For this review, use the dimensioned drawing (mm, ordinates from the lowest corner) and the shaded views. A direction names the side the tool comes from. Round coordinates to 2 decimals unless told otherwise and drop trailing zeros. Order: outer loops, then holes, each group sorted by start corner. A loop starts at its lowest first (then second) coordinate and runs counter-clockwise, first axis right, second up. Notation, with made-up numbers: M 47.5,-18.5 L 90.5,-18.5 A23 ccw 90.5,5.5 Z; hole C 31.25,36.5 d9. An arc over 180 degrees is marked long. One line per item, written item: value. Start each with the question number.
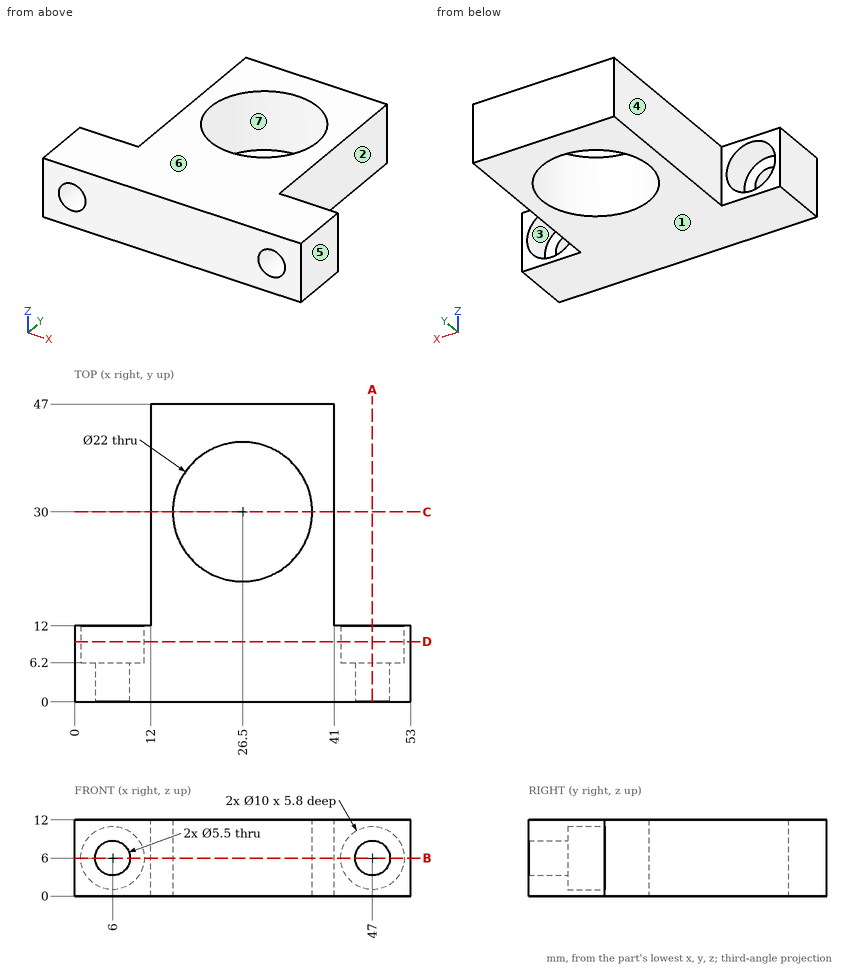
Item 1: The part is to be moulded in two halves that separate along X. For the marked faces 4, 5, 6 and 7, say which applies: pulls with the +X half, pulls with the -X half, needs draft (parallel to the pull), parting line crosses it, or undercut.
Item 2: Consider section A-A, the plane x = 47. Give the boundary of the cut face in (y, z), then the cut area to 3 significant figures.
Item 3: Machinability: for the marked faces 1, 2 and 3, which of the approach directions +Z, -Z, +X, -X, +Y, -Y give a long, thin tool a straight path to every point of the face, cutting with its end or side? Answer none if there is none.
Item 4: Consider section D-D, the plane y = 9.5. Give the boundary of the cut face in (x, z), then the cut area to 3 significant figures.
Item 5: Wall thickness on L1, parallel to Y at x = 26.5, z = 3; L2, parallel to Z at x = 47, y = 1.5; L3, parallel to X at y = 4, z = 8.25: over which ranges is each line inside the solid? List them lowest first.
Item 6: Consider section B-B, the plane z = 6. Give the boundary of the cut face in (x, y).
Item 7: Consider section C-C, the plane y = 30. Give the boundary of the cut face in (x, z), then the cut area to 3 significant figures.
Item 8: Clearance check with flat-ended pins moving along their axes: P1, Ø6, axis at x = 47, z = 6, coming from the -Y side; P2, Ø1.5, axis at x = 43.5, z = 9, coming from the +Y side; P3, Ø3.5, axis at x = 6, z = 6, coming from the +Y side (3 decimals); P4, Ø3.5, axis at y = 31, z = 7.5, coming from the +X side. State where each tip first meets the part, or that it passes through.
Computed:
1. face 4: pulls with the -X half
1. face 5: pulls with the +X half
1. face 6: needs draft
1. face 7: undercut
2. outline: M 0,0 L 12,0 L 12,1 L 6.2,1 L 6.2,3.25 L 0,3.25 Z; M 0,8.75 L 6.2,8.75 L 6.2,11 L 12,11 L 12,12 L 0,12 Z
2. area: 51.9 mm^2
3. face 1: -Z, +X, -X, +Y, -Y
3. face 2: +Z, -Z, +X, +Y
3. face 3: +Y
4. outline: M 0,0 L 53,0 L 53,12 L 0,12 Z; hole C 6,6 d10; hole C 47,6 d10
4. area: 479 mm^2
5. L1: y = 0 to 19, 41 to 47
5. L2: z = 0 to 3.25, 8.75 to 12
5. L3: x = 0 to 4.42, 7.58 to 45.42, 48.58 to 53
6. outline: M 0,0 L 3.25,0 L 3.25,6.2 L 1,6.2 L 1,12 L 0,12 Z; M 8.75,0 L 44.25,0 L 44.25,6.2 L 42,6.2 L 42,12 L 41,12 L 41,47 L 12,47 L 12,12 L 11,12 L 11,6.2 L 8.75,6.2 Z; M 49.75,0 L 53,0 L 53,12 L 52,12 L 52,6.2 L 49.75,6.2 Z; hole C 26.5,30 d22
7. outline: M 12,0 L 15.5,0 L 15.5,12 L 12,12 Z; M 37.5,0 L 41,0 L 41,12 L 37.5,12 Z
7. area: 84.0 mm^2
8. P1: stops at y = 0
8. P2: stops at y = 12
8. P3: passes through
8. P4: stops at x = 41
